Geometry check sheet. Reference: the model listing, model coordinates, mm. Face numbers are marked on the shaded views. Round coordinates to 2 decimals unless told otherwise and drop trailing zeros. Loops run counter-clockwise (first coordinate to the right, second up) from the corner with the lowest first, then second, coordinate; pieces in that order, holes last. Notation, with made-up numbers: (20.5, -26) -> (44.5, -26) arc R25 cw to (44.5, 1) -> close; hole circle Ø10 at (3, 33.25). An arc over 180 degrees is marked (long way). Use a Markdown table: item, result. Add a question column.
Q1. Material ranges on L1, parallel to Y at x = 0, z = 23; L2, parallel to Y at x = 1.5, z = 28.5; L3, parallel to X at y = -5, z = 18.5 (3 decimals), recorded low to high.
Q2. Release check for a two-part mould opening along X. For the marked faces 1, 2 and 3 record: released by +X, released by -X, zero draft, split by the parting line, or undercut.
Q3. Sectioned sample at C-C, the plane z = 5. Enter the section's corners in (x, y), then the cut area to 3 significant figures.
Q4. Gauge pin test, flat ends, axial feed: P1, Ø3, axis at x = 6, y = 6, coming from the +Z side; P2, Ø4, axis at x = -5, z = 15.5, coming from the -Y side; P3, Ø2, axis at y = 4.5, z = 9.5, coming from the -X side; P4, Ø6, axis at x = 5, z = 15, coming from the +Y side. Record the tip position at first contact, or that the pin passes through.
Q5. Sectioned sample at A-A, the plane x = 0. Enter the section's corners in (y, z).
```python
from build123d import *

# Parameters (mm, degrees)
SKETCH1_R           = 8
SKETCH1_R_2         = 6.25
BOSS_EXTRUDE1_DEPTH = 50
SKETCH2_W           = 20.877121254
SKETCH2_H           = 20.159055414
SKETCH2_W_2         = 15.8
SKETCH2_H_2         = 15.8
CUT_EXTRUDE1_DEPTH  = 50


with BuildPart() as part:
    # Sketch1 → Boss-Extrude1 (new body)
    with BuildSketch(Plane.XY):
        Circle(SKETCH1_R)
        Circle(SKETCH1_R_2, mode=Mode.SUBTRACT)
    extrude(amount=BOSS_EXTRUDE1_DEPTH)

    # Sketch2 → Cut-Extrude1 (cut)
    with BuildSketch(Plane.XY.offset(50)):
        Rectangle(SKETCH2_W, SKETCH2_H)
        Rectangle(SKETCH2_W_2, SKETCH2_H_2, mode=Mode.SUBTRACT)
    extrude(amount=-CUT_EXTRUDE1_DEPTH, mode=Mode.SUBTRACT)


solid = part.part
```
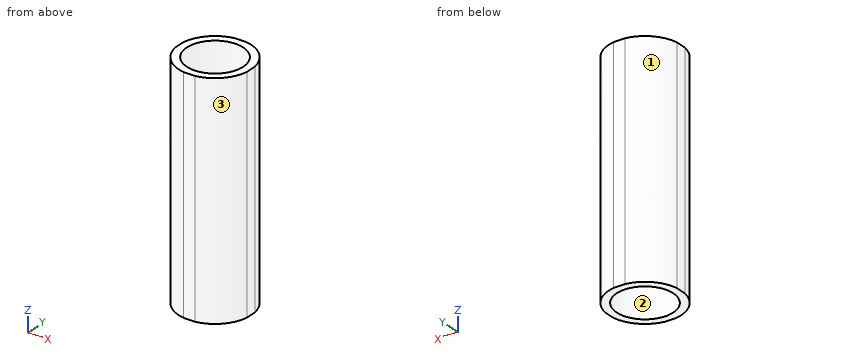
Values:
| question | item | result |
|---|---|---|
| 1 | L1 | -7.9 to -6.25, 6.25 to 7.9 |
| 1 | L2 | -7.86 to -6.07, 6.07 to 7.86 |
| 1 | L3 | -6.245 to -3.75, 3.75 to 6.245 |
| 2 | face 1 | released by -X |
| 2 | face 2 | undercut |
| 2 | face 3 | released by +X |
| 3 | outline | (-7.9, -1.26) arc R8 ccw to (-1.26, -7.9) -> (1.26, -7.9) arc R8 ccw to (7.9, -1.26) -> (7.9, 1.26) arc R8 ccw to (1.26, 7.9) -> (-1.26, 7.9) arc R8 ccw to (-7.9, 1.26) -> close; hole circle Ø12.5 at (0, 0) |
| 3 | area | 77.7 mm^2 |
| 4 | P1 | z = 50 |
| 4 | P2 | y = -7.42 |
| 4 | P3 | x = -7.19 |
| 4 | P4 | y = 7.75 |
| 5 | outline | (-7.9, 0) -> (-6.25, 0) -> (-6.25, 50) -> (-7.9, 50) -> close; (6.25, 0) -> (7.9, 0) -> (7.9, 50) -> (6.25, 50) -> close |
